Check sheet for the drawn part. Datum: minimum x, y, z corner. Units: mm. A direction names the side the tool comes from. Coordinates: 2 decimals unless noted, no trailing zeros. Loops run counter-clockwise (first coordinate to the right, second up) from the corner with the lowest first, then second, coordinate; pieces in that order, holes last. Notation, with made-up numbers: (0.25, 71) - (15.25, 71) arc R11 ccw to (15.25, 82) - close; hole circle Ø2 at (35.25, 75.25). An arc over 180 degrees is marked (long way). Write item = value, one per line. Start each with the question number.
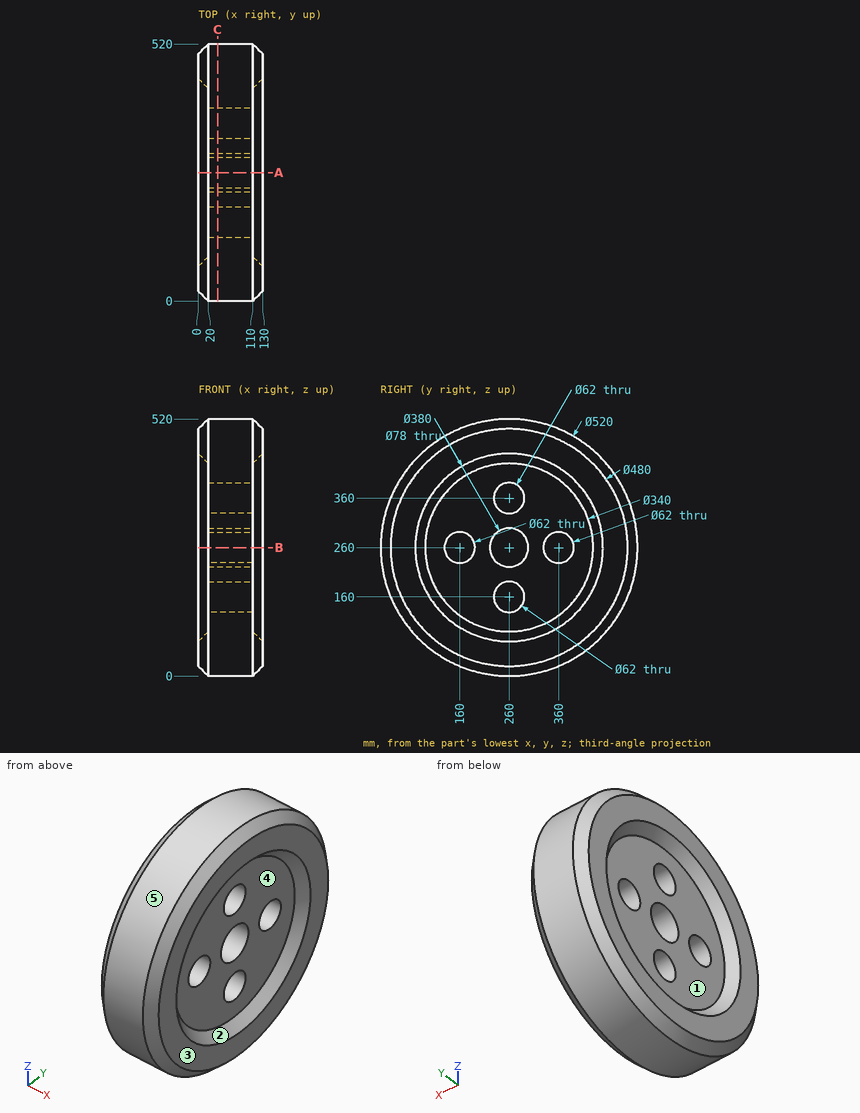
(1) Sectioned sample at C-C on x = 39. Enter the section's corners in (y, z), plus the area to 3 significant figures.
(2) Draft check along Z on the marked faces 3, 4 and 5. Enter one of: pulls with the +Z half, pulls with the -Z half, needs draft (parallel to the pull), parting line crosses it, or undercut.
(3) Scan lines: line 1 (Y direction, x = 90.5, z = 260); line 2 (Y direction, x = 68, z = 360); line 3 (Y direction, x = 99, z = 263.5). Record each from-to range of solid material in increasing order.
(4) Sectioned sample at A-A on y = 260. Enter the section's corners in (x, z).
(5) Depth check by flat-ended pin: pin 1 (5 mm diameter, centred on y = 100, z = 461.5, fed in from +X); pin 2 (3 mm diameter, centred on x = 37.5, z = 208, fed in from -Y); pin 3 (2 mm diameter, centred on y = 297.5, z = 105, fed in from -X). Enter the tip coordinate at first touch or a pass-through.
(6) Tool access check on the marked faces 1 and 2. Record the directions out of +Z, -Z, +X, -X, +Y, -Y that give a thin tool (end or side, any length) a straight path to the whole face; none if there is none.
Working result:
q1.outline = circle Ø520 at (260, 260); hole circle Ø62 at (160, 260); hole circle Ø78 at (260, 260); hole circle Ø62 at (260, 160); hole circle Ø62 at (260, 360); hole circle Ø62 at (360, 260)
q1.area = 196,000 mm2
q2.face_3 = needs draft
q2.face_4 = undercut
q2.face_5 = parting line crosses it
q3.line_1 = 0 to 129, 191 to 221, 299 to 329, 391 to 520
q3.line_2 = 20 to 229, 291 to 500
q3.line_3 = 0.02 to 129.2, 190.8 to 221.16, 298.84 to 329.2, 390.8 to 519.98
q4.outline = (0, 20) - (20, 0) - (110, 0) - (130, 20) - (130, 70) - (110, 90) - (110, 129) - (20, 129) - (20, 90) - (0, 70) - close; (0, 450) - (20, 430) - (20, 391) - (110, 391) - (110, 430) - (130, 450) - (130, 500) - (110, 520) - (20, 520) - (0, 500) - close; (20, 191) - (110, 191) - (110, 221) - (20, 221) - close; (20, 299) - (110, 299) - (110, 329) - (20, 329) - close
q5.pin_1 = 115.2
q5.pin_2 = 4.95
q5.pin_3 = 20
q6.face_1 = -X
q6.face_2 = +X
